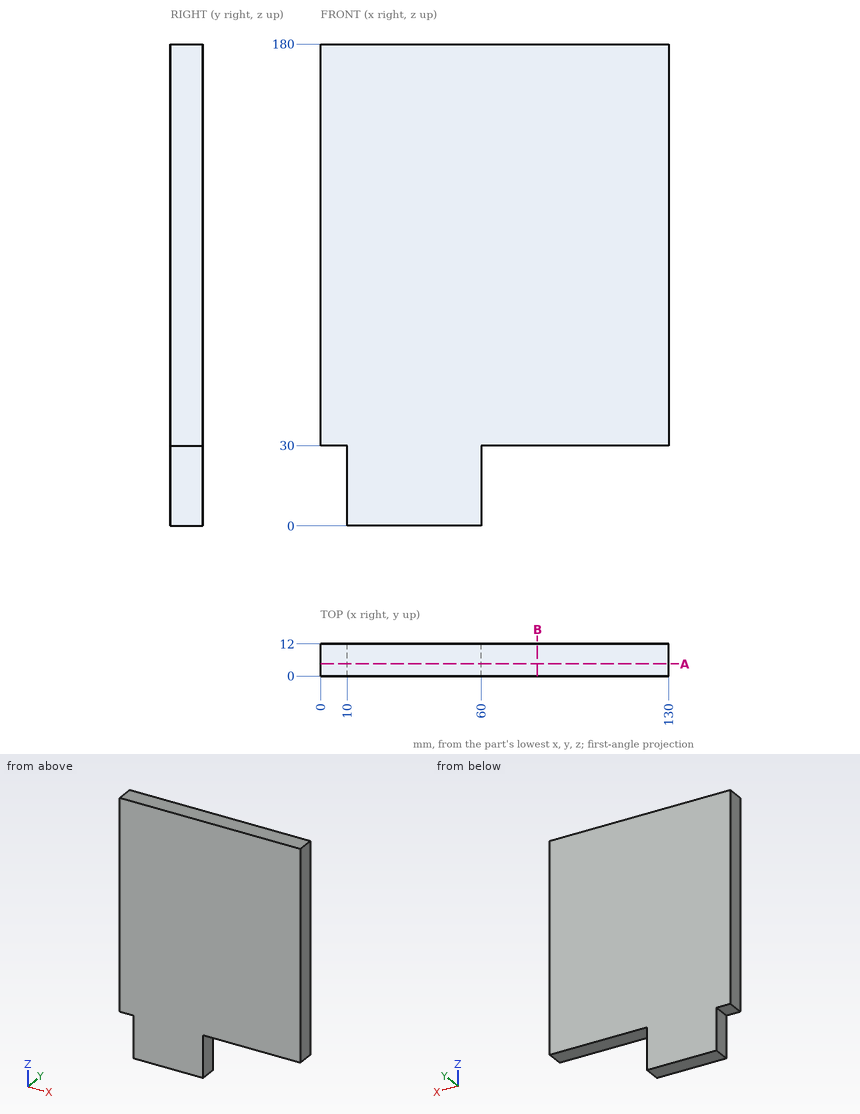
Answer from the drawing. Dimensions are ordinates in mm from the lowest x, y and z of the part. Coordinates: 2 decimals unless noted, no trailing zeros. Loops run counter-clockwise (first coordinate to the right, second up) from the corner with the lowest first, then second, coordinate; pieces in that order, holes last.
1) Flat-ended cylindrical pins translate along their axes: pin 1 (3 mm diameter, centred on x = 26, y = 8, fed in from -Z); pin 2 (1.5 mm diameter, centred on y = 9.5, z = 25.5, fed in from -X); pin 3 (6 mm diameter, centred on x = 85, y = 8.5, fed in from -Z). Find the tip coordinate at first contact, or state that the pin passes through.
Results:
pin 1: stops at z = 0
pin 2: stops at x = 10
pin 3: stops at z = 30
2) Consider probe 1 along Z at (x, y) = (95, 2); probe 2 along X at (y, z) = (9, 23). Determine where each line is inside the solid, lowest interval first.
Results:
probe 1: z = 30 to 180
probe 2: x = 10 to 60
3) Section B-B (x = 81) is taken. Give the vertices of the cut face in (y, z), plus the area to 3 significant figures.
Results:
outline: (0, 30) - (12, 30) - (12, 180) - (0, 180) - close
area: 1,800 mm2
4) Section A-A (y = 4.5) is taken. Give the vertices of the cut face in (x, z).
Results:
outline: (0, 30) - (10, 30) - (10, 0) - (60, 0) - (60, 30) - (130, 30) - (130, 180) - (0, 180) - close
